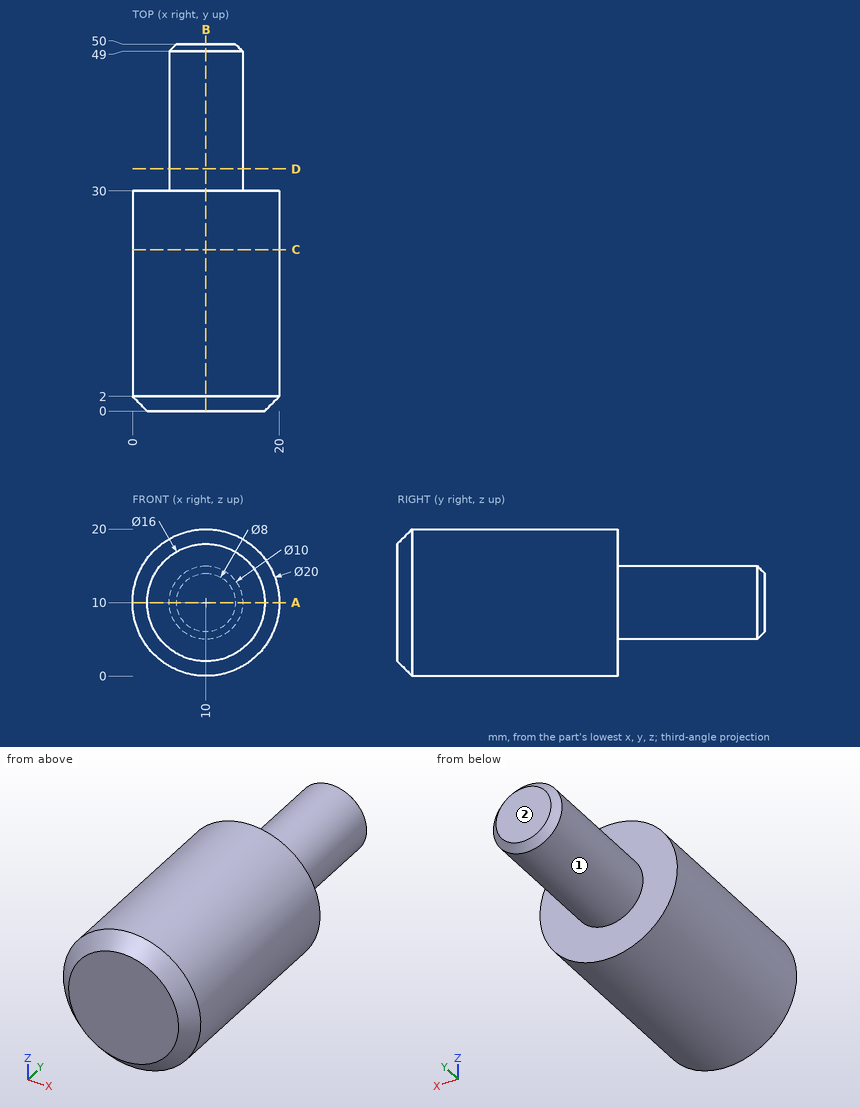
Part print with two shaded views. Sizes in mm from the minimum x, y, z corner. A direction names the side the tool comes from. Round coordinates to 2 decimals unless told otherwise and drop trailing zeros. Write each loop counter-clockwise with the first axis right and the second up, starting at its lowest first coordinate (ties: lowest second). Pieces come first, ordered by that corner, then holes. Notation, with made-up numbers: (-31, -35) -> (23, -35) arc R20 ccw to (23, -24) -> close; hole circle Ø1 at (-27, -7). An arc over 180 degrees is marked (long way). Put each result on its own line as item: value.
Item 1: Slice it at B-B, the plane x = 10. Give the cut face in (y, z), plus the area to 3 significant figures.
Here are the results:
outline: (0, 2) -> (2, 0) -> (30, 0) -> (30, 5) -> (49, 5) -> (50, 6) -> (50, 14) -> (49, 15) -> (30, 15) -> (30, 20) -> (2, 20) -> (0, 18) -> close
area: 795 mm^2
Item 2: Tool access for the marked faces 1 and 2: list every direction of +Z, -Z, +X, -X, +Y, -Y with a clear straight run to the whole face (end or side of a thin tool).
Here are the results:
face 1: +Y
face 2: +Z, -Z, +X, -X, +Y
Item 3: Slice it at A-A, the plane z = 10. Give the cut face in (x, y), plus the area to 3 significant figures.
Here are the results:
outline: (0, 2) -> (2, 0) -> (18, 0) -> (20, 2) -> (20, 30) -> (15, 30) -> (15, 49) -> (14, 50) -> (6, 50) -> (5, 49) -> (5, 30) -> (0, 30) -> close
area: 795 mm^2
Item 4: Flat gauge pins, fed straight in: P1, Ø6, axis at x = 16, y = 34, coming from the -Z side; P2, Ø12, axis at x = 15, y = 38.5, coming from the +Z side; P3, Ø1, axis at x = 6.5, y = 24.5, coming from the -Z side. Where does each tip first touch, or does it go through?
Here are the results:
P1: stops at z = 6
P2: stops at z = 15
P3: stops at z = 0.46
Item 5: Slice it at D-D, the plane y = 33. Give the cut face in (x, z).
Here are the results:
outline: circle Ø10 at (10, 10)
Item 6: Wall check: probe 1 along Y at (x, z) = (5.75, 13.5); probe 2 along X at (y, z) = (3, 10); probe 3 along Y at (x, z) = (19, 9.5). Give the ranges that are in metal, low to high. Write a range as from..to.
Here are the results:
probe 1: y = 0..30
probe 2: x = 0..20
probe 3: y = 1.01..30
Item 7: Slice it at C-C, the plane y = 22. Give the cut face in (x, z).
Here are the results:
outline: circle Ø20 at (10, 10)
